Design review of the part built by this model. Coordinates are the model's own, in mm. A direction names the side the tool comes from. Coordinates: 2 decimals unless noted, no trailing zeros. Loops run counter-clockwise (first coordinate to the right, second up) from the corner with the lowest first, then second, coordinate; pieces in that order, holes last. Notation, with made-up numbers: M 78.5,60 L 104.5,60 A33 cw 104.5,95 Z; hole C 84,48.5 d5. An arc over 180 degrees is marked long. Answer as a JSON object with one key per item and string values. Group by question number.
1. Consider section A-A (x = 113.5). State the section outline as (y, z) points.
2. Consider section C-C (z = -26). State the section outline as (x, y) points.
3. Draft analysis for pull direction Y (two halves, no side actions). For faces 1 (the flat face through (125, 8, -30)), 2 (the cylindrical face through (16.872, 50.233, -0.238)), 3 (the flat face through (61.625, 10.084, -40.749)), 4 (the flat face through (62, 0, -15)), state which applies: +Y half, -Y half, draft (parallel to the pull), parting line (faces both ways), or undercut.
4. Consider section B-B (y = 34). Count the separate pieces of the cut face and the enclosed holes in it, then the cut area to 3 significant figures.
5. To check wall thickness, follow probe 1 along Y at (x, z) = (118.5, -33.5); probe 2 along Z at (x, y) = (10, 22.5); probe 3 along Y at (x, z) = (15, -5). State the ranges of each line that lie inside material, in increasing order.
6. Insertion check: pin 1 (4 mm diameter, centred on x = 13.5, y = 78.5, fed in from +Z); pin 2 (17 mm diameter, centred on x = 47.64, y = 31, fed in from -Z); pin 3 (1.5 mm diameter, centred on y = 69, z = 8, fed in from -X); pin 4 (8 mm diameter, centred on x = 19.87, y = 56, fed in from +Z). Each pin has a flat end and moves straight along its axis. Give the tip position at first contact, or say it passes through.
7. Machinability: for faces 5 (the flat face through (62.68, 44.37, -8.32)), 6 (the flat face through (9, 77, 7)), 7 (the flat face through (42, 22, 18)), which of the approach directions +Z, -Z, +X, -X, +Y, -Y give a long, thin tool a straight path to every point of the face, cutting with its end or side? Answer none if there is none.
from build123d import *

# Parameters (mm, degrees)
TRIANGULAR_BRACKET_BODY_DEPTH    = 18
RECTANGULAR_CUT_15X56_DEPTH      = 11
HOLE_SKETCH_R                    = 6
HOLE_CUT_DEPTH                   = 11
SLIDE_RAIL_125_DEPTH             = 125
RAIL_GROOVE_SKETCH_R             = 6.5
RAIL_GROOVE_CUT_DEPTH            = 125
RECTANGULAR_CUT_CHAMFER_1MM_SIZE = 1
HOLE_AND_GROOVE_CHAMFER_1MM_SIZE = 1
BODY_EDGE_FILLET_R2_A_R          = 2
BODY_EDGE_FILLET_R2_B_R          = 2


with BuildPart() as part:
    # Bracket Profile Sketch → Triangular Bracket Body (new, symmetric)
    with BuildSketch(Plane.XY):
        Polygon((0, 0), (111.955126335, 0), (12, 90), (0, 90), align=None)
    extrude(amount=TRIANGULAR_BRACKET_BODY_DEPTH, both=True)

    # Rectangular Cut Sketch → Rectangular Cut 15x56 (cut)
    with BuildSketch(Plane.XY.offset(18)):
        Polygon((23.147172382, 79.963040905), (0, 56), (0, 90), (12, 90), align=None)
    extrude(amount=-RECTANGULAR_CUT_15X56_DEPTH, mode=Mode.SUBTRACT)

    # Hole Sketch → Hole Cut (cut)
    with BuildSketch(Plane(origin=(50.126314512, 55.670912219, 0), x_dir=(0.743144825477398, -0.669130606358854, 0), z_dir=(0.669130606358854, 0.743144825477398, 0))):
        with Locations(Location((16.198872821, 0, 0), (0, 0, 180))):
            Circle(HOLE_SKETCH_R)
    extrude(amount=-HOLE_CUT_DEPTH, mode=Mode.SUBTRACT)

    # Slide Rail Profile Sketch → Slide Rail 125 (add)
    with BuildSketch(Plane.ZY):
        Polygon((-18, 16), (-33.698956889, 16), (-48, 4), (-48, 0), (-18, 0), align=None)
    extrude(amount=-SLIDE_RAIL_125_DEPTH)

    # Rail Groove Sketch → Rail Groove Cut (cut)
    with BuildSketch(Plane(origin=(0, 0, -18), x_dir=(-1, 0, 0), z_dir=(0, 0, -1))):
        with Locations((-47.636607378, 31)):
            Circle(RAIL_GROOVE_SKETCH_R)
        with Locations((-19.871294507, 56)):
            Circle(RAIL_GROOVE_SKETCH_R)
    extrude(amount=-RAIL_GROOVE_CUT_DEPTH, mode=Mode.SUBTRACT)

    # Rectangular Cut Chamfer 1mm
    rectangular_cut_chamfer_1mm_edges = [part.edges().sort_by_distance(p)[0] for p in [
        (11.573586191, 67.981520452, 18),
    ]]
    chamfer(rectangular_cut_chamfer_1mm_edges, length=RECTANGULAR_CUT_CHAMFER_1MM_SIZE)

    # Hole and Groove Chamfer 1mm
    hole_and_groove_chamfer_1mm_edges = [part.edges().sort_by_distance(p)[0] for p in [
        (66.623291981, 40.816966988, 0),
        (54.136607378, 31, 18),
        (54.136607378, 31, -18),
        (26.371294507, 56, 18),
        (26.371294507, 56, -18),
    ]]
    chamfer(hole_and_groove_chamfer_1mm_edges, length=HOLE_AND_GROOVE_CHAMFER_1MM_SIZE)

    # Body Edge Fillet R2 A
    body_edge_fillet_r2_a_edges = [part.edges().sort_by_distance(p)[0] for p in [
        (53.092663049, 53, -18),
    ]]
    fillet(body_edge_fillet_r2_a_edges, radius=BODY_EDGE_FILLET_R2_A_R)

    # Body Edge Fillet R2 B
    body_edge_fillet_r2_b_edges = [part.edges().sort_by_distance(p)[0] for p in [
        (67.92295004, 39.646749615, 18),
    ]]
    fillet(body_edge_fillet_r2_b_edges, radius=BODY_EDGE_FILLET_R2_B_R)


solid = part.part
Findings below:
{
 "1": {"outline": "M 0,-48 L 4,-48 L 16,-33.7 L 16,-18 L 0,-18 Z"},
 "2": {"outline": "M 0,0 L 125,0 L 125,16 L 0,16 Z"},
 "3": {"face 1": "draft", "face 2": "undercut", "face 3": "+Y half", "face 4": "-Y half"},
 "4": {"separate pieces": "2", "enclosed holes": "1", "area": "2,230 mm^2"},
 "5": {"probe 1": "y = 0 to 16", "probe 2": "z = -18 to 18", "probe 3": "y = 0 to 51.7, 60.3 to 87.3"},
 "6": {"pin 1": "stops at z = 7", "pin 2": "stops at z = -18", "pin 3": "stops at x = 11.83", "pin 4": "passes through"},
 "7": {"face 5": "+Z, +X, +Y", "face 6": "+Z, -X, +Y", "face 7": "+Z, +X, -X, +Y, -Y"}
}
